from build123d import *

# Parameters (mm, degrees)
HEX_BODY_67AF_X16_DEPTH = 16
COLLAR_PROFILE_56_R     = 28
COLLAR_56_X16_DEPTH     = 16
BORE_PROFILE_12_5_R     = 6.25
BORE_12_5_THROUGH_DEPTH = 61.353817885


with BuildPart() as part:
    # Hex Profile 67AF → Hex Body 67AF x16 (new body)
    with BuildSketch(Plane(origin=(0, 0, 0), x_dir=(1, 0, 0), z_dir=(0, 1, 0))):
        Polygon((0, -38.682468036), (33.5, -19.341234018), (33.5, 19.341234018), (0, 38.682468036), (-33.5, 19.341234018), (-33.5, -19.341234018), align=None)
    extrude(amount=HEX_BODY_67AF_X16_DEPTH)

    # Collar Profile Ø56 → Collar Ø56 x16 (add)
    with BuildSketch(Plane.XZ):
        with Locations(Location((0, 0, 0), (0, 0, 270))):
            Circle(COLLAR_PROFILE_56_R)
    extrude(amount=COLLAR_56_X16_DEPTH)

    # Bore Profile Ø12.5 → Bore Ø12.5 Through (cut, through all)
    with BuildSketch(Plane.XZ.offset(16)):
        with Locations(Location((0, 0, 0), (0, 0, 270))):
            Circle(BORE_PROFILE_12_5_R)
    extrude(amount=-BORE_12_5_THROUGH_DEPTH, mode=Mode.SUBTRACT)


solid = part.part
Input: part model. Units: mm. Frame: model coordinates. A direction names the side the tool comes from. Give positions to 0.01 mm unless a question says otherwise; leave off trailing zeros. Write each loop counter-clockwise with the first axis right and the second up, starting at its lowest first coordinate (ties: lowest second). Pieces come first, ordered by that corner, then holes. Notation, with made-up numbers: M 80.5,-24 L 88.5,-24 A25 cw 88.5,-3 Z; hole C 89,29 d2. An arc over 180 degrees is marked long. Use one line per item in the form item = value.
1. Cut plane D-D on z = -27. Return loops of the section in (x, y), and give its area (3 significant figures).
Outcome:
outline = M -20.23,0 L -7.42,0 L -7.42,-16 L 7.42,-16 L 7.42,0 L 20.23,0 L 20.23,16 L -20.23,16 Z
area = 885 mm²
2. Cut plane B-B on z = 0. Return loops of the section in (x, y).
Outcome:
outline = M -33.5,0 L -28,0 L -28,-16 L -6.25,-16 L -6.25,16 L -33.5,16 Z; M 6.25,-16 L 28,-16 L 28,0 L 33.5,0 L 33.5,16 L 6.25,16 Z
3. Cut plane C-C on x = -5. Return loops of the section in (y, z).
Outcome:
outline = M -16,-27.55 L 0,-27.55 L 0,-35.8 L 16,-35.8 L 16,-3.75 L -16,-3.75 Z; M -16,3.75 L 16,3.75 L 16,35.8 L 0,35.8 L 0,27.55 L -16,27.55 Z
4. First-contact query: P1, Ø2, axis at y = 10, z = -23.5, coming from the -X side; P2, Ø5, axis at y = 10, z = 19.5, coming from the +X side; P3, Ø6, axis at y = -8.5, z = -26.5, coming from the -X side; P4, Ø12, axis at x = -26.5, y = -4, coming from the +Z side. Flat tips, straight axial feed; report the tip coordinate or a pass-through.
Outcome:
P1 = -28.03
P2 = 33.5
P3 = -15.22
P4 = 25.96
5. Mould query, pull axis X, two halves, no side actions, for faces 3 (the face through (16.516, 7.888, 29.147)), 4 (the face through (-16.516, 7.888, -29.147)), 5 (the face through (1.88, -0.22, -5.96)). Classes: released by +X, released by -X, zero draft, split by the parting line, or undercut.
Outcome:
face_3 = released by +X
face_4 = released by -X
face_5 = undercut
6. Reachability of faces 1 (the face through (-27.334, -7.888, 6.07)), 2 (the face through (-33.5, 8, 0)) from +Z, -Z, +X, -X, +Y, -Y: full face, straight path, thin tool, end or side. Return the list, or none.
Outcome:
face_1 = -Y
face_2 = +Z, -Z, -X, +Y, -Y
7. Cut plane A-A on y = 5.5. Return loops of the section in (x, z), and give its area (3 significant figures).
Outcome:
outline = M -33.5,-19.34 L 0,-38.68 L 33.5,-19.34 L 33.5,19.34 L 0,38.68 L -33.5,19.34 Z; hole C 0,0 d12.5
area = 3,760 mm²
8. Ray query, L1, parallel to X at y = 7, z = 0; L2, parallel to X at y = -1, z = 0; L3, parallel to Z at x = -18.5, y = 4. Return the intervals inside material, ascending.
Outcome:
L1 = -33.5 to -6.25, 6.25 to 33.5
L2 = -28 to -6.25, 6.25 to 28
L3 = -28 to 28
